from build123d import *

# Parameters (mm, degrees)
MOUNTING_TAB_PROFILE_R               = 2.65
MOUNTING_TAB_1MM_WITH_HOLE_5_3_DEPTH = 1
CHAMBER_BODY_PROFILE_19_R            = 9.5
CHAMBER_BODY_19X19_DEPTH             = 19
TOP_PIN_PROFILE_5_R                  = 2.5
TOP_PIN_5X4_DEPTH                    = 4


with BuildPart() as part:
    # Mounting Tab Profile → Mounting Tab 1mm with Hole Ø5.3 (new body)
    with BuildSketch(Plane(origin=(0, 0, 0), x_dir=(1, 0, 0), z_dir=(0, 1, 0))):
        with BuildLine():
            Line((-4.5, 8), (4.5, 8))
            ThreePointArc((4.5, 8), (12.5, 0), (4.5, -8))
            Line((4.5, -8), (-4.5, -8))
            ThreePointArc((-4.5, -8), (-12.5, 0), (-4.5, 8))
        make_face()
        with Locations(Location((4.5, 0, 0), (0, 0, 270))):
            Circle(MOUNTING_TAB_PROFILE_R, mode=Mode.SUBTRACT)
    extrude(amount=MOUNTING_TAB_1MM_WITH_HOLE_5_3_DEPTH)

    # Chamber Body Profile Ø19 → Chamber Body Ø19x19 (add)
    with BuildSketch(Plane(origin=(0, 1, 0), x_dir=(1, 0, 0), z_dir=(0, 1, 0))):
        with Locations(Location((-12.5, 0, 0), (0, 0, 53.576426358))):
            Circle(CHAMBER_BODY_PROFILE_19_R)
    extrude(amount=CHAMBER_BODY_19X19_DEPTH)

    # Top Pin Profile Ø5 → Top Pin Ø5x4 (add)
    with BuildSketch(Plane(origin=(0, 20, 0), x_dir=(1, 0, 0), z_dir=(0, 1, 0))):
        with Locations(Location((-12.5, 0, 0), (0, 0, 270))):
            Circle(TOP_PIN_PROFILE_5_R)
    extrude(amount=TOP_PIN_5X4_DEPTH)


solid = part.part
Source: CAD feature listing. Evaluate the final solid. Frame: model axes, mm. A direction names the side the tool comes from. Round coordinates to 2 decimals unless told otherwise and drop trailing zeros. Loops run counter-clockwise (first coordinate to the right, second up) from the corner with the lowest first, then second, coordinate; pieces in that order, holes last. Notation, with made-up numbers: M 78,-29 L 111,-29 A30 ccw 111,1 Z; hole C 70.25,22.5 d9. An arc over 180 degrees is marked long. Return JSON: item names as keys, results as strings. Group by question number.
1. Section query B-B on x = -3.5. Output: boundary loops of the cut face in (y, z), and give its area (3 significant figures).
2. Mould query, pull axis Z, two halves, no side actions, for faces 4 (the face through (-12, 24, 0)), 5 (the face through (0.1, 0.5, 8)), 6 (the face through (1.91, 0.49, -0.57)). Classes: released by +Z, released by -Z, zero draft, split by the parting line, or undercut.
3. Section query A-A on z = 0. Output: boundary loops of the cut face in (x, y).
4. Material intervals for line 1 along X through (y, z) = (0.7, 0); line 2 along Y through (x, z) = (8.5, -0.5); line 3 along Y through (x, z) = (-10, 2), sorted ascending. Write a range as from..to.
5. Reachability of faces 1 (the face through (-12.498, 0.493, 0.176)), 2 (the face through (12.498, 0.493, -0.176)), 3 (the face through (-14.94, 21.97, -0.54)) from +Z, -Z, +X, -X, +Y, -Y: full face, straight path, thin tool, end or side. Return the list, or none.
6. Section query C-C on z = 4.5. Output: boundary loops of the cut face in (x, y).
7. Section query D-D on y = 8.25. Output: boundary loops of the cut face in (x, z).
8. Pin query (flat end, axial travel): pin 1 (2 mm diameter, centred on x = -5.5, y = 5, fed in from +Z); pin 2 (4 mm diameter, centred on x = -3.5, y = 6, fed in from +Z); pin 3 (1.1 mm diameter, centred on x = -2, y = 0.5, fed in from +Z); pin 4 (8 mm diameter, centred on y = 6, z = -0.5, fed in from -X). Return the tip coordinate at first contact, or that it passes through.
Checks:
{
 "1": {"outline": "M 0,-8 L 1,-8 L 1,-3.04 L 20,-3.04 L 20,3.04 L 1,3.04 L 1,8 L 0,8 Z", "area": "132 mm²"},
 "2": {"face 4": "zero draft", "face 5": "released by +Z", "face 6": "undercut"},
 "3": {"outline": "M -22,1 L -12.5,1 L -12.5,0 L 1.85,0 L 1.85,1 L -3,1 L -3,20 L -10,20 L -10,24 L -15,24 L -15,20 L -22,20 Z; M 7.15,0 L 12.5,0 L 12.5,1 L 7.15,1 Z"},
 "4": {"line 1": "x = -12.5..1.85, 7.15..12.5", "line 2": "y = 0..1", "line 3": "y = 0..20"},
 "5": {"face 1": "-X, -Y", "face 2": "+X, +Y, -Y", "face 3": "+Y"},
 "6": {"outline": "M -20.87,1 L -11.11,1 L -11.11,0 L 11.11,0 L 11.11,1 L -4.13,1 L -4.13,20 L -20.87,20 Z"},
 "7": {"outline": "C -12.5,0 d19"},
 "8": {"pin 1": "stops at z = 7.37", "pin 2": "stops at z = 6.42", "pin 3": "stops at z = 8", "pin 4": "stops at x = -22"}
}
